Model file for the job. Use its own axes, mm. A direction names the side the tool comes from. Give positions to 0.01 mm unless a question says otherwise; leave off trailing zeros. Write each loop counter-clockwise with the first axis right and the second up, starting at its lowest first coordinate (ties: lowest second). Pieces come first, ordered by that corner, then holes. Notation, with made-up numbers: M 25,-3 L 44,-3 A25 cw 44,35 Z; hole C 70,3 d4. An arc over 180 degrees is marked long. Answer as a JSON object with one key per item and string values. Group by question number.
```python
from build123d import *

# Parameters (mm, degrees)
SKETCH_1_R      = 5
EXTRUDE_4_DEPTH = 10


with BuildPart() as part:
    # 草图1 → 凸台-拉伸4 (new body)
    with BuildSketch(Plane.XY):
        Polygon((0, 125), (-10.24210316, 107.26015695), (-23.656405545, 122.741087158), (-30.356133186, 103.383495415), (-46.457806958, 116.045991627), (-49.373013467, 95.770284992), (-67.580102182, 105.156691604), (-66.605424401, 84.695686942), (-86.259876435, 90.466754763), (-81.430541758, 70.559966093), (-101.821994006, 72.507113696), (-93.312547172, 53.874024228), (-113.703999419, 51.926876625), (-101.821994006, 35.24093476), (-121.47644604, 29.469866939), (-106.651328683, 15.33414609), (-124.858417398, 5.947739478), (-107.626006464, -5.126858572), (-123.727680235, -17.789354784), (-104.710799954, -25.402565207), (-118.125102339, -40.883495415), (-98.011072313, -44.76015695), (-108.253175473, -62.5), (-87.768969153, -62.5), (-94.468696794, -81.857591743), (-74.354666768, -77.980930207), (-77.269873278, -98.256636843), (-58.252992997, -90.64342642), (-57.278315216, -111.104431082), (-40.045904282, -100.029833032), (-35.216569605, -119.936621702), (-20.391452248, -105.800900853), (-11.882005413, -124.433990322), (0, -107.748048456), (11.882005413, -124.433990322), (20.391452248, -105.800900853), (35.216569605, -119.936621702), (40.045904282, -100.029833032), (57.278315216, -111.104431082), (58.252992997, -90.64342642), (77.269873278, -98.256636843), (74.354666768, -77.980930207), (94.468696794, -81.857591743), (87.768969153, -62.5), (108.253175473, -62.5), (98.011072313, -44.76015695), (118.125102339, -40.883495415), (104.710799954, -25.402565207), (123.727680235, -17.789354784), (107.626006464, -5.126858572), (124.858417398, 5.947739478), (106.651328683, 15.33414609), (121.47644604, 29.469866939), (101.821994006, 35.24093476), (113.703999419, 51.926876625), (93.312547172, 53.874024228), (101.821994006, 72.507113696), (81.430541758, 70.559966093), (86.259876435, 90.466754763), (66.605424401, 84.695686942), (67.580102182, 105.156691604), (49.373013467, 95.770284992), (46.457806958, 116.045991627), (30.356133186, 103.383495415), (23.656405545, 122.741087158), (10.24210316, 107.26015695), align=None)
        Circle(SKETCH_1_R, mode=Mode.SUBTRACT)
    extrude(amount=EXTRUDE_4_DEPTH)


solid = part.part
```
Q1. 3-axis set-ups, long thin cutter, end or side, ignore diameter. For faces 1 (the flat face through (75.833, -88.261, 4.93)), 2 (the flat face through (113.96, 22.303, 4.93)), 3 (the flat face through (37.6, -110.12, 4.93)), 4 (the flat face through (-103.366, 52.914, 4.93)): which of +Z, -Z, +X, -X, +Y, -Y reach the whole face in a straight line?
Q2. Two-plate mould, pull along X, no slides. Class faces 5 (the flat face through (103.651, 52.887, 4.93)), 6 (the flat face through (-47.895, 106.05, 4.93)), 7 (the flat face through (-115.627, 10.707, 4.93)), 8 (the flat face through (67.086, 94.783, 4.93)): +X half, -X half, draft (parallel to the pull), parting line (faces both ways), or undercut.
Q3. Slice it at A-A, the plane y = 0. Write the cut outline in (x, z), then the cut area to 3 significant figures.
Q4. Wall check: L1, parallel to Y at x = 0, z = 3; L2, parallel to Y at x = -109.5, z = 6; L3, parallel to X at y = 112, z = 4.75. Give the ranges that are in metal, low to high.
Q5. Drop flat-ended pins along their axis: P1, Ø2, axis at y = 78.5, z = 3, coming from the -X side; P2, Ø3, axis at x = -67, z = 3, coming from the +Y side; P3, Ø3, axis at x = -87, z = 6, coming from the +Y side; P4, Ø9, axis at x = 0, y = 0, coming from the -Z side. Give the stop position or say it passes through.
Q6. Slice it at B-B, the plane y = 46. Write the cut outline in (x, z).
Solved:
{
 "1": {"face 1": "+Z, -Z", "face 2": "+Z, -Z, +X", "face 3": "+Z, -Z, -Y", "face 4": "+Z, -Z, -X"},
 "2": {"face 5": "+X half", "face 6": "undercut", "face 7": "-X half", "face 8": "undercut"},
 "3": {"outline": "M -115.6,0 L -5,0 L -5,10 L -115.6,10 Z; M 5,0 L 115.6,0 L 115.6,10 L 5,10 Z", "area": "2,210 mm²"},
 "4": {"L1": "y = -107.75 to -5, 5 to 125", "L2": "y = -42.55 to -30.93, -23.49 to -6.6, -3.92 to 13.87, 18.05 to 32.99, 46.02 to 52.33", "L3": "x = -47.04 to -41.31, -27.37 to -14.35, -7.51 to 7.51, 14.35 to 27.37, 41.31 to 47.04"},
 "5": {"P1": "stops at x = -83.6", "P2": "stops at y = 105.16", "P3": "stops at y = 90.47", "P4": "passes through"},
 "6": {"outline": "M -109.48,0 L 109.48,0 L 109.48,10 L -109.48,10 Z"}
}
